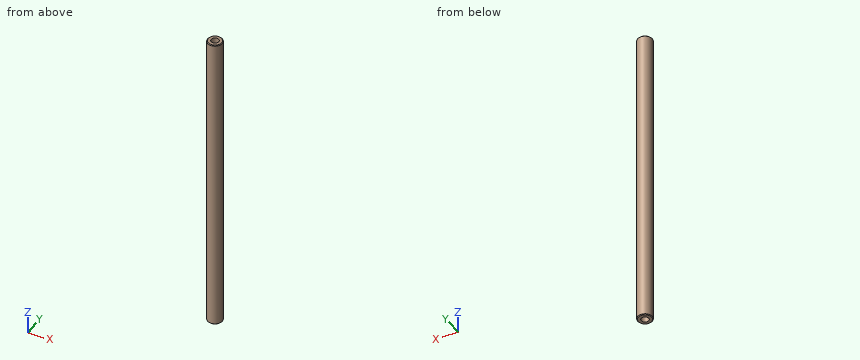
```python
from build123d import *

# Parameters (mm, degrees)
HOLE_WIZARD_M12_5_D     = 10.2
HOLE_WIZARD_M12_5_DEPTH = 220
HOLE_WIZARD_M12_5_TIP   = 3.064389157
HOLE_WIZARD_M12_6_D     = 10.2
HOLE_WIZARD_M12_6_DEPTH = 220
HOLE_WIZARD_M12_6_TIP   = 3.064389157


with BuildPart() as part:
    # 草图1 → 旋转1 (revolve)
    with BuildSketch(Plane.XZ, mode=Mode.PRIVATE) as revolve_1_sk:
        Polygon((9, -207.5), (10, -206.5), (10, 206.5), (9, 207.5), (0, 207.5), (0, -207.5), align=None)
    revolve(revolve_1_sk.sketch.rotate(Axis((0, 0, 207.5), (0, 0, -1)), 180), axis=Axis((0, 0, 207.5), (0, 0, -1)))

    # M12 螺纹孔5
    with Locations(Plane(origin=(0, 0, -207.5), x_dir=(-1, 0, 0), z_dir=(0, 0, -1))):
        with Locations((0, 0)):
            Hole(HOLE_WIZARD_M12_5_D / 2, depth=HOLE_WIZARD_M12_5_DEPTH)
            with Locations((0, 0, -(HOLE_WIZARD_M12_5_DEPTH + HOLE_WIZARD_M12_5_TIP / 2))):  # 118° drill point
                Cone(0, HOLE_WIZARD_M12_5_D / 2, HOLE_WIZARD_M12_5_TIP, mode=Mode.SUBTRACT)

    # M12 螺纹孔6
    with Locations(Plane.XY.offset(207.5)):
        with Locations((0, 0)):
            Hole(HOLE_WIZARD_M12_6_D / 2, depth=HOLE_WIZARD_M12_6_DEPTH)
            with Locations((0, 0, -(HOLE_WIZARD_M12_6_DEPTH + HOLE_WIZARD_M12_6_TIP / 2))):  # 118° drill point
                Cone(0, HOLE_WIZARD_M12_6_D / 2, HOLE_WIZARD_M12_6_TIP, mode=Mode.SUBTRACT)


solid = part.part
```
The model under review builds one solid part; all positions refer to its coordinate system, in mm. Give positions to 0.01 mm unless a question says otherwise; leave off trailing zeros. Write each loop counter-clockwise with the first axis right and the second up, starting at its lowest first coordinate (ties: lowest second). Pieces come first, ordered by that corner, then holes. Notation, with made-up numbers: M 32,-3 L 69,-3 A10 cw 69,15 Z; hole C -32,61 d6. An arc over 180 degrees is marked long. Write item = value, one per line. Start each with the question number.
Q1. Clearance check with flat-ended pins moving along their axes: pin 1 (9 mm diameter, centred on x = 0, y = 0, fed in from -Z); pin 2 (6 mm diameter, centred on x = -6, z = -149.5, fed in from -Y); pin 3 (1 mm diameter, centred on x = 5, z = 25.5, fed in from -Y). State where each tip first meets the part, or that it passes through.
Q2. We need section A-A (x = 0). State the section outline as (y, z) points, plus the area to 4 significant figures.
Q3. For line 1 (Y direction, x = 0, z = -152.5); line 2 (Y direction, x = -0.75, z = -56); line 3 (X direction, y = 2, z = -30.5), list the stretches that pass through material, from the lowest coordinate up.
Result set:
q1.pin_1 = through
q1.pin_2 = -9.54
q1.pin_3 = -8.93
q2.outline = M -10,-206.5 L -9,-207.5 L -5.1,-207.5 L -5.1,207.5 L -9,207.5 L -10,206.5 Z; M 5.1,-207.5 L 9,-207.5 L 10,-206.5 L 10,206.5 L 9,207.5 L 5.1,207.5 Z
q2.area = 4,065 mm2
q3.line_1 = -10 to -5.1, 5.1 to 10
q3.line_2 = -9.97 to -5.04, 5.04 to 9.97
q3.line_3 = -9.8 to -4.69, 4.69 to 9.8
